from build123d import *

# Parameters (mm, degrees)
BOSS_EXTRUDE1_DEPTH = 300
SKETCH2_R           = 4.5
CUT_EXTRUDE1_DEPTH  = 300
CUT_EXTRUDE2_DEPTH  = 300
CHAMFER1_SIZE       = 5
FILLET1_R           = 2
FILLET2_R           = 10


with BuildPart() as part:
    # Sketch1 → Boss-Extrude1 (new body)
    with BuildSketch(Plane.XY):
        Polygon((0, 0), (0, -90), (128, -90), (128, -82), (8, -82), (8, 0), align=None)
    extrude(amount=BOSS_EXTRUDE1_DEPTH)

    # Sketch2 → Cut-Extrude1 (cut)
    with BuildSketch(Plane(origin=(0, -82, 0), x_dir=(1, 0, 0), z_dir=(0, 1, 0))):
        with Locations(Location((63, -12.5, 0), (0, 0, 270))):
            Circle(SKETCH2_R)
        with Locations(Location((113, -12.5, 0), (0, 0, 270))):
            Circle(SKETCH2_R)
        with Locations(Location((63, -287.5, 0), (0, 0, 270))):
            Circle(SKETCH2_R)
        with Locations(Location((113, -287.5, 0), (0, 0, 270))):
            Circle(SKETCH2_R)
    extrude(amount=-CUT_EXTRUDE1_DEPTH, mode=Mode.SUBTRACT)

    # Sketch3 → Cut-Extrude2 (cut)
    with BuildSketch(Plane(origin=(8, 0, 0), x_dir=(0, 0, -1), z_dir=(1, 0, 0))):
        with BuildLine():
            Line((-270.5, -12), (-270.5, -62))
            ThreePointArc((-270.5, -62), (-275, -66.5), (-279.5, -62))
            Line((-279.5, -62), (-279.5, -12))
            ThreePointArc((-279.5, -12), (-275, -7.5), (-270.5, -12))
        make_face()
        with BuildLine():
            Line((-29.5, -12), (-29.5, -62))
            ThreePointArc((-29.5, -62), (-25, -66.5), (-20.5, -62))
            Line((-20.5, -62), (-20.5, -12))
            ThreePointArc((-20.5, -12), (-25, -7.5), (-29.5, -12))
        make_face()
    extrude(amount=-CUT_EXTRUDE2_DEPTH, mode=Mode.SUBTRACT)

    # Chamfer1
    chamfer1_edges = [part.edges().sort_by_distance(p)[0] for p in [
        (4, 0, 300),
        (4, 0, 0),
        (128, -86, 0),
        (128, -86, 300),
    ]]
    chamfer(chamfer1_edges, length=CHAMFER1_SIZE)

    # Fillet1
    fillet1_edges = [part.edges().sort_by_distance(p)[0] for p in [
        (8, -82, 150),
    ]]
    fillet(fillet1_edges, radius=FILLET1_R)

    # Fillet2
    fillet2_edges = [part.edges().sort_by_distance(p)[0] for p in [
        (0, -90, 150),
    ]]
    fillet(fillet2_edges, radius=FILLET2_R)


solid = part.part
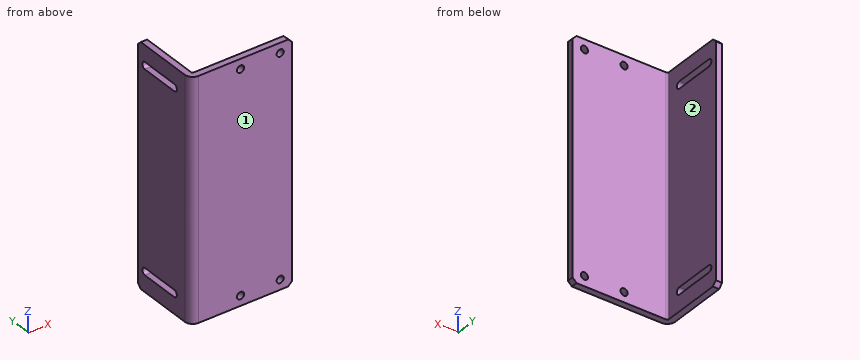
Geometry: final body of the model. Coordinates: model frame, mm. Face numbers are marked on the shaded views. A direction names the side the tool comes from. Give positions to 0.01 mm unless a question says otherwise; leave off trailing zeros. Write each loop counter-clockwise with the first axis right and the second up, starting at its lowest first coordinate (ties: lowest second). Pieces come first, ordered by that corner, then holes. Notation, with made-up numbers: M 13.25,64 L 58.25,64 A22 ccw 58.25,73 Z; hole C 82.25,71.25 d8. An arc over 180 degrees is marked long. Answer in a Markdown table with one row per item. Add a question column.
(1) Ray query, line 1 (X direction, y = -85, z = 287); line 2 (X direction, y = -84.25, z = 12.5); line 3 (Y direction, x = 26, z = 105.5). Return the intervals inside material, ascending.
(2) Section A-A on z = 12.5. Return loops of the section in (x, y).
(3) Section C-C on y = -41.5. Return loops of the section in (x, z), and give its area (3 significant figures).
(4) Section B-B on x = 113. Return loops of the section in (y, z).
(5) First-contact query: pin 1 (7 mm diameter, centred on x = 113, z = 12.5, fed in from +Y); pin 2 (11.5 mm diameter, centred on x = 113, z = 287.5, fed in from +Y). Flat tips, straight axial feed; report the tip coordinate or a pass-through.
(6) Reachability of the marked faces 1 and 2 from +Z, -Z, +X, -X, +Y, -Y: full face, straight path, thin tool, end or side. Return the list, or none.
(7) Section D-D on z = 96. Return loops of the section in (x, y).
Result set:
| question | item | result |
|---|---|---|
| 1 | line 1 | x = 1.34 to 58.53, 67.47 to 108.53, 117.47 to 128 |
| 1 | line 2 | x = 0.95 to 58.5, 67.5 to 108.5, 117.5 to 128 |
| 1 | line 3 | y = -90 to -82 |
| 2 | outline | M 0,-80 A10 ccw 10,-90 L 58.5,-90 L 58.5,-82 L 10,-82 A2 cw 8,-80 L 8,0 L 0,0 Z; M 67.5,-90 L 108.5,-90 L 108.5,-82 L 67.5,-82 Z; M 117.5,-90 L 128,-90 L 128,-82 L 117.5,-82 Z |
| 3 | outline | M 0,0 L 8,0 L 8,20.5 L 0,20.5 Z; M 0,29.5 L 8,29.5 L 8,270.5 L 0,270.5 Z; M 0,279.5 L 8,279.5 L 8,300 L 0,300 Z |
| 3 | area | 2,260 mm^2 |
| 4 | outline | M -90,0 L -82,0 L -82,8 L -90,8 Z; M -90,17 L -82,17 L -82,283 L -90,283 Z; M -90,292 L -82,292 L -82,300 L -90,300 Z |
| 5 | pin 1 | passes through |
| 5 | pin 2 | stops at y = -82 |
| 6 | face 1 | +Z, -Z, +X, -X, -Y |
| 6 | face 2 | +Z, -Z, +X, +Y |
| 7 | outline | M 0,-80 A10 ccw 10,-90 L 128,-90 L 128,-82 L 10,-82 A2 cw 8,-80 L 8,0 L 0,0 Z |
